```python
from build123d import *

# Parameters (mm, degrees)
C_BRACKET_BODY_DEPTH = 5
FLANGE_HOLE_SKETCH_R = 1.5
FLANGE_HOLES_3_DEPTH = 100
WEB_HOLE_SKETCH_R    = 2.5
WEB_HOLE_DEPTH       = 100


with BuildPart() as part:
    # C Profile Sketch → C Bracket Body (new, symmetric)
    with BuildSketch(Plane.XY):
        Polygon((0, 0), (0, 28), (9, 37), (25, 37), (25, 32), (22, 32), (22, 34), (14, 34), (14, 32), (11.071067812, 32), (5, 25.928932188), (5, 5), (14, 5), (14, 3), (22, 3), (22, 5), (25, 5), (25, 0), align=None)
    extrude(amount=C_BRACKET_BODY_DEPTH, both=True)

    # Flange Hole Sketch → Flange Holes Ø3 (cut, symmetric)
    with BuildSketch(Plane.XZ.offset(-34)):
        with Locations(Location((18, 0, 0), (0, 0, 270))):
            Circle(FLANGE_HOLE_SKETCH_R)
    extrude(amount=FLANGE_HOLES_3_DEPTH, both=True, mode=Mode.SUBTRACT)

    # Web Hole Sketch → Web Hole (cut, symmetric)
    with BuildSketch(Plane(origin=(5, 0, 0), x_dir=(0, 0, -1), z_dir=(1, 0, 0))):
        with Locations((0, 12)):
            Circle(WEB_HOLE_SKETCH_R)
    extrude(amount=WEB_HOLE_DEPTH, both=True, mode=Mode.SUBTRACT)


solid = part.part
```
For this review, take the finished solid that the model builds, in its own axes (mm). A direction names the side the tool comes from. Round coordinates to 2 decimals unless told otherwise and drop trailing zeros. Loops run counter-clockwise (first coordinate to the right, second up) from the corner with the lowest first, then second, coordinate; pieces in that order, holes last.
(1) Mouldability with a two-part tool opening along X and no side actions: class faces 4 (the flat face through (20, 34, 0)), 5 (the flat face through (9, 5, 0)), 6 (the flat face through (0, 14, 2)) as released by +X, released by -X, zero draft, split by the parting line, or undercut.
Returned:
face 4: undercut
face 5: zero draft
face 6: released by -X
(2) Clearance check with flat-ended pins moving along their axes: P1, Ø6, axis at y = 11.5, z = -0.5, coming from the +X side; P2, Ø1.6, axis at y = 33, z = -0.5, coming from the -X side; P3, Ø10, axis at x = 18, y = 24.5, coming from the +Z side. State where each tip first meets the part, or that it passes through.
Returned:
P1: stops at x = 5
P2: stops at x = 4.2
P3: passes through
(3) Tool access review of faces 1 (the flat face through (16, 3, 0)), 2 (the flat face through (5, 16, 0)), 3 (the flat face through (15, 37, 0)): name each direction out of +Z, -Z, +X, -X, +Y, -Y from which nothing blocks a thin tool from reaching the whole face with its end or side.
Returned:
face 1: +Z, -Z
face 2: +Z, -Z, +X
face 3: +Z, -Z, +X, -X, +Y
(4) Wall thickness on line 1 along Y through (x, z) = (16.75, 2.5); line 2 along X through (y, z) = (1.4, 0); line 3 along Y through (x, z) = (11.25, -3.5): over which ranges is each line inside the solid? List them lowest first.
Returned:
line 1: y = 0 to 3, 34 to 37
line 2: x = 0 to 16.5, 19.5 to 25
line 3: y = 0 to 5, 32 to 37
(5) We need section A-A (x = 18). Give the boundary of the cut face in (y, z).
Returned:
outline: (0, -5) - (3, -5) - (3, -1.5) - (0, -1.5) - close; (0, 1.5) - (3, 1.5) - (3, 5) - (0, 5) - close; (34, -5) - (37, -5) - (37, -1.5) - (34, -1.5) - close; (34, 1.5) - (37, 1.5) - (37, 5) - (34, 5) - close
(6) We need section C-C (y = 12). Give the boundary of the cut face in (x, z).
Returned:
outline: (0, -5) - (5, -5) - (5, -2.5) - (0, -2.5) - close; (0, 2.5) - (5, 2.5) - (5, 5) - (0, 5) - close
(7) We need section D-D (x = 15.5). Give the boundary of the cut face in (y, z), plus the area to 3 significant figures.
Returned:
outline: (0, -5) - (3, -5) - (3, 5) - (0, 5) - close; (34, -5) - (37, -5) - (37, 5) - (34, 5) - close
area: 60.0 mm2
(8) We need section B-B (z = 2). Give the boundary of the cut face in (x, y).
Returned:
outline: (0, 0) - (25, 0) - (25, 5) - (22, 5) - (22, 3) - (14, 3) - (14, 5) - (5, 5) - (5, 10.5) - (0, 10.5) - close; (0, 13.5) - (5, 13.5) - (5, 25.93) - (11.07, 32) - (14, 32) - (14, 34) - (22, 34) - (22, 32) - (25, 32) - (25, 37) - (9, 37) - (0, 28) - close
